```python
from build123d import *

# Parameters (mm, degrees)
BOSS_EXTRUDE1_DEPTH = 3.2


with BuildPart() as part:
    # Sketch1 → Boss-Extrude1 (new body)
    with BuildSketch(Plane(origin=(0, 0, 0), x_dir=(0, 0, -1), z_dir=(1, 0, 0))):
        Polygon((-4, 2.309401077), (-4, -2.309401077), (0, -4.618802154), (4, -2.309401077), (4, 2.309401077), (0, 4.618802154), align=None)
    extrude(amount=BOSS_EXTRUDE1_DEPTH)

    # Sketch2 → Cut-Revolve1 (revolve, cut)
    with BuildSketch(Plane.XY):
        Polygon((0, 4), (1.6, 6.771281292), (3.2, 4), (3.2, 10.2), (0, 10.2), align=None)
    revolve(axis=Axis((50, 0, 0), (-1, 0, 0)), mode=Mode.SUBTRACT)

    # Sketch3 → Cut-Revolve2 (revolve, cut)
    with BuildSketch(Plane.XY, mode=Mode.PRIVATE) as cut_revolve2_sk:
        Polygon((0, 0), (0, 2.5), (0.433, 2.067), (2.767, 2.067), (3.2, 2.5), (3.2, 0), align=None)
    revolve(cut_revolve2_sk.sketch.rotate(Axis((3.2, 0, 0), (-1, 0, 0)), 90), axis=Axis((3.2, 0, 0), (-1, 0, 0)), mode=Mode.SUBTRACT)


solid = part.part
```
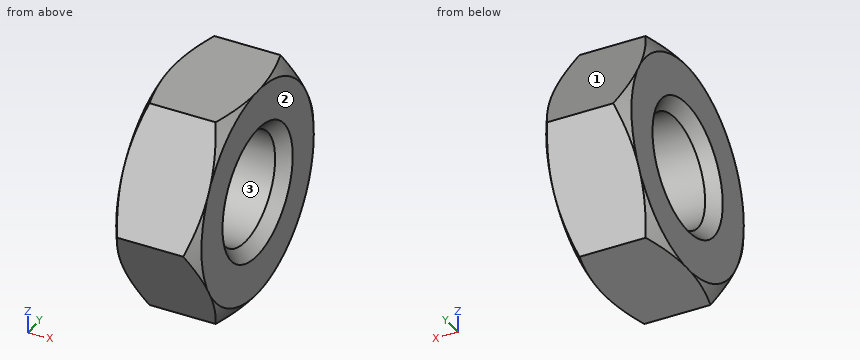
The listing builds one solid part. Answer for the finished solid, in the listing's coordinates (mm). Face numbers are marked on the shaded views. Coordinates: 2 decimals unless noted, no trailing zeros. Write each loop counter-clockwise with the first axis right and the second up, starting at its lowest first coordinate (ties: lowest second). Pieces come first, ordered by that corner, then holes. Notation, with made-up numbers: (3, 79) - (49, 79) arc R21 ccw to (49, 89) - close; hole circle Ø5 at (2, 16). An arc over 180 degrees is marked (long way). Return JSON: item names as keys, results as strings. Group by question number.
1. Straight lines are drawn through the part: L1, parallel to Y at x = 0.35, z = 0.75; L2, parallel to Z at x = 1.5, y = -0.25; L3, parallel to Y at x = 1.25, z = -1.25. For each, find the intervals that lie inside material, in ascending order.
2. A cutting plane is placed at A-A, the plane x = 1.8. Determine the outline of the cut face in (y, z), plus the area to 3 significant figures.
3. Determine the mould class of the marked faces 1, 2 and 3 for opening direction Y: released by +Y, released by -Y, zero draft, split by the parting line, or undercut.
4. Given pin 1 (1.5 mm diameter, centred on y = 2.5, z = 3, fed in from -X); pin 2 (2 mm diameter, centred on y = 0.5, z = -1, fed in from -X), each flat-ended and moving along its own axis, determine where each tip first touches the part or whether it passes through.
Ans:
{
 "1": {"L1": "-4.19 to -2.01, 2.01 to 4.19", "L2": "-4 to -2.05, 2.05 to 4", "L3": "-3.9 to -1.65, 1.65 to 3.9"},
 "2": {"outline": "(-4.62, 0) - (-2.31, -4) - (2.31, -4) - (4.62, 0) - (2.31, 4) - (-2.31, 4) - close; hole circle Ø4.13 at (0, 0)", "area": "42.0 mm²"},
 "3": {"face 1": "released by +Y", "face 2": "zero draft", "face 3": "undercut"},
 "4": {"pin 1": "x = 0", "pin 2": "x = 0.38"}
}
